```python
from build123d import *

# Parameters (mm, degrees)
SKETCH1_R           = 1.5
BOSS_EXTRUDE1_DEPTH = 3


with BuildPart() as part:
    # Sketch1 → Boss-Extrude1 (new body)
    with BuildSketch(Plane.XY):
        with BuildLine():
            Line((0, 3), (45, 3))
            ThreePointArc((45, 3), (48, 0), (45, -3))
            Line((45, -3), (0, -3))
            ThreePointArc((0, -3), (-3, 0), (0, 3))
        make_face()
        Circle(SKETCH1_R, mode=Mode.SUBTRACT)
        with Locations((45, 0)):
            Circle(SKETCH1_R, mode=Mode.SUBTRACT)
    extrude(amount=BOSS_EXTRUDE1_DEPTH)


solid = part.part
```
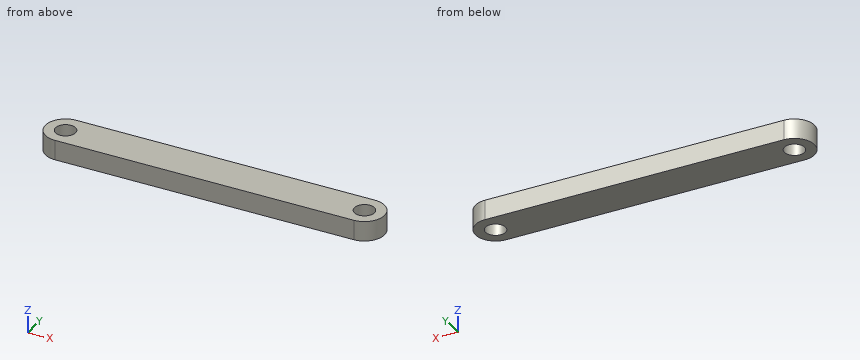
The model under review builds one solid part; all positions refer to its coordinate system, in mm. Round coordinates to 2 decimals unless told otherwise and drop trailing zeros. Order: outer loops, then holes, each group sorted by start corner. A loop starts at its lowest first (then second) coordinate and runs counter-clockwise, first axis right, second up.
(1) Wall thickness on L1, parallel to Y at x = 0, z = 1.2; L2, parallel to X at y = 0.4, z = 2.05; L3, parallel to X at y = -1.35, z = 2.85: over which ranges is each line inside the solid? List them lowest first.
Working result:
L1: y = -3 to -1.5, 1.5 to 3
L2: x = -2.97 to -1.45, 1.45 to 43.55, 46.45 to 47.97
L3: x = -2.68 to -0.65, 0.65 to 44.35, 45.65 to 47.68
(2) Take a section at A-A, the plane y = 0. State the section outline as (x, z) points.
Working result:
outline: (-3, 0) - (-1.5, 0) - (-1.5, 3) - (-3, 3) - close; (1.5, 0) - (43.5, 0) - (43.5, 3) - (1.5, 3) - close; (46.5, 0) - (48, 0) - (48, 3) - (46.5, 3) - close
(3) For P1, Ø2.5, axis at x = 45, y = 0, coming from the -Z side, flat-tipped, find the tip position at first contact; note if it passes through.
Working result:
P1: passes through
(4) Take a section at B-B, the plane z = 2. State the section outline as (x, y) points, plus the area to 3 significant figures.
Working result:
outline: (0, -3) - (45, -3) arc R3 ccw to (45, 3) - (0, 3) arc R3 ccw to start; hole circle Ø3 at (0, 0); hole circle Ø3 at (45, 0)
area: 284 mm2
